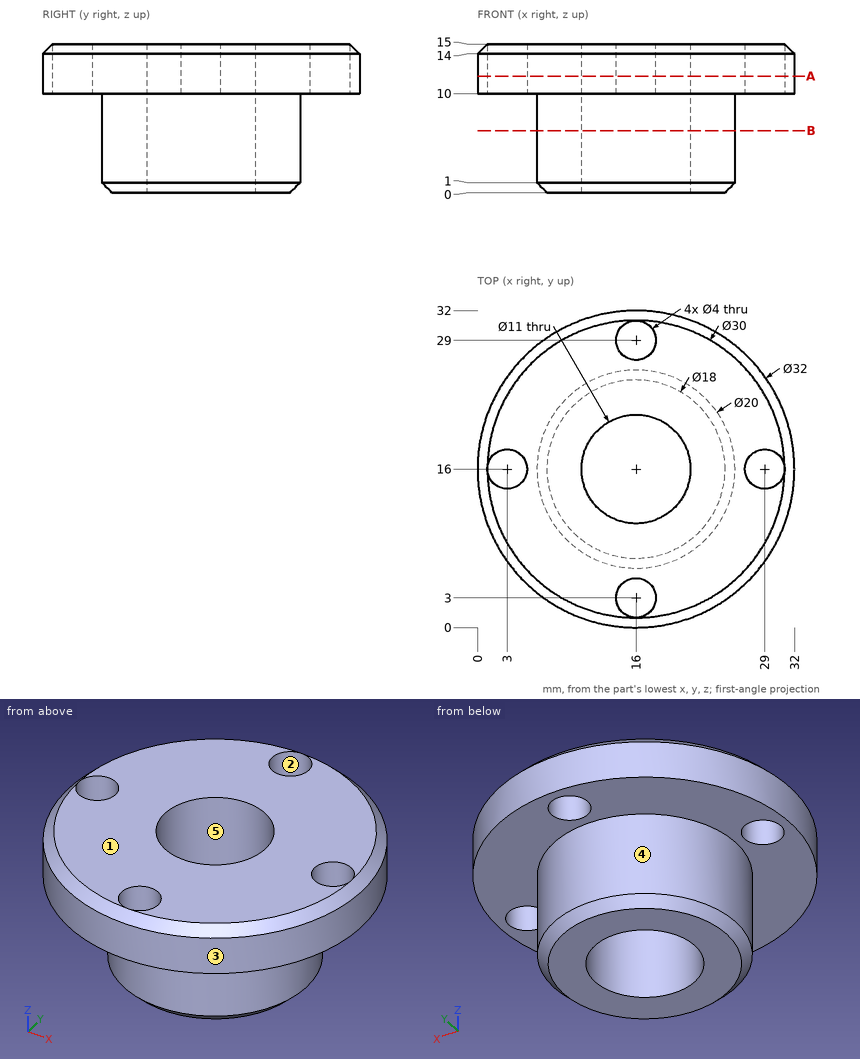
Check sheet for the drawn part. Datum: minimum x, y, z corner. Units: mm. A direction names the side the tool comes from. Round coordinates to 2 decimals unless told otherwise and drop trailing zeros. Order: outer loops, then holes, each group sorted by start corner. A loop starts at its lowest first (then second) coordinate and runs counter-clockwise, first axis right, second up.
1) Go/stop test with flat-tipped pins: pin 1 Ø5 at (x, y) = (17.5, 28) entering from -Z; pin 2 Ø6.5 at (x, y) = (16, 16) entering from -Z; pin 3 Ø8 at (y, z) = (3.5, 9) entering from +X; pin 4 Ø6 at (x, z) = (24.5, 9) entering from -Y. Record where each tip stops, or that it passes through.
2) Section check A-A (z = 11.75). Record the boundary of the cut face in (x, y), and give its area (3 significant figures).
3) Section check B-B (z = 6.25). Record the boundary of the cut face in (x, y).
4) Mould release check, pull along X, two halves, no side actions. Record for the marked faces 1, 2 and 3: +X half, -X half, draft (parallel to the pull), parting line (faces both ways), or undercut.
5) Tool access check on the marked faces 4 and 5. Record the directions out of +Z, -Z, +X, -X, +Y, -Y that give a thin tool (end or side, any length) a straight path to the whole face; none if there is none.
6) Scan lines: line 1 (Y direction, x = 16, z = 12.95); line 2 (Z direction, x = 3.5, y = 10.5); line 3 (X direction, y = 18.5, z = 11.5). Record each from-to range of solid material in increasing order.
Result:
1. pin 1: stops at z = 0.59
1. pin 2: passes through
1. pin 3: stops at x = 29.47
1. pin 4: stops at y = 1.04
2. outline: circle Ø32 at (16, 16); hole circle Ø4 at (3, 16); hole circle Ø11 at (16, 16); hole circle Ø4 at (16, 3); hole circle Ø4 at (16, 29); hole circle Ø4 at (29, 16)
2. area: 659 mm2
3. outline: circle Ø20 at (16, 16); hole circle Ø11 at (16, 16)
4. face 1: draft
4. face 2: undercut
4. face 3: parting line
5. face 4: -Z
5. face 5: +Z, -Z
6. line 1: y = 0 to 1, 5 to 10.5, 21.5 to 27, 31 to 32
6. line 2: z = 10 to 15
6. line 3: x = 0.2 to 11.1, 20.9 to 31.8
